```python
from build123d import *

# Parameters (mm, degrees)
BRACKET_PLATE_PROFILE_R    = 9
BRACKET_PLATE_PROFILE_R_2  = 4
BRACKET_PLATE_PROFILE_R_3  = 6
BRACKET_PLATE_8MM_DEPTH    = 8
ARMS_70MM_DEPTH            = 70
GUSSET_TAPER_CUT_PROFILE_R = 6
GUSSET_TAPER_CUT_DEPTH     = 50
ARM_TRIM_CUT_PROFILE_R     = 4
ARM_TRIM_CUT_DEPTH         = 50


with BuildPart() as part:
    # Bracket Plate Profile → Bracket Plate 8mm (new body)
    with BuildSketch(Plane.XY):
        with BuildLine():
            Line((-48.472135955, 36.092742474), (-14.562305899, -10.580134541))
            ThreePointArc((-14.562305899, -10.580134541), (-5.562305899, -17.119017293), (5.562305899, -17.119017293))
            Line((5.562305899, -17.119017293), (85.708203932, 8.92196355))
            ThreePointArc((85.708203932, 8.92196355), (93.852260087, 22.211855326), (82, 32.334641746))
            Line((82, 32.334641746), (8.459892396, 32.334641746))
            ThreePointArc((8.459892396, 32.334641746), (0.445914591, 33.106300041), (-7.273584527, 35.392919854))
            Line((-7.273584527, 35.392919854), (-39.003147253, 48.212495329))
            ThreePointArc((-39.003147253, 48.212495329), (-48.304086029, 45.720316295), (-48.472135955, 36.092742474))
        make_face()
        Circle(BRACKET_PLATE_PROFILE_R, mode=Mode.SUBTRACT)
        with Locations((-42, 40.795024493)):
            Circle(BRACKET_PLATE_PROFILE_R_2, mode=Mode.SUBTRACT)
        with Locations((82, 20.334641746)):
            Circle(BRACKET_PLATE_PROFILE_R_3, mode=Mode.SUBTRACT)
    extrude(amount=BRACKET_PLATE_8MM_DEPTH)

    # Arm Sections 34x6 → Arms 70mm (add)
    with BuildSketch(Plane.XY.offset(8)):
        Polygon((37.898227453, -6.612439485), (43.604566551, -4.758337518), (32.307498994, 30.01046132), (26.601159896, 28.156359354), align=None)
        Polygon((-38.07371599, 21.780545234), (-34.547004477, 16.926443267), (-12.049603456, 33.271761878), (-15.57631497, 38.125863845), align=None)
    extrude(amount=ARMS_70MM_DEPTH)

    # Gusset Taper Cut Profile → Gusset Taper Cut (cut)
    with BuildSketch(Plane(origin=(38.042260652, 12.360679775, 0), x_dir=(0, 0, -1), z_dir=(0.9510565162951532, 0.30901699437494873, 0))):
        with BuildLine():
            Line((-50.49494029, 9.525500165), (-8, 18.558078561))
            Line((-8, 18.558078561), (-78, 18.558078561))
            Line((-78, 18.558078561), (-78, -18))
            Line((-78, -18), (-8, -18))
            Line((-8, -18), (-8, -14.212271044))
            Line((-8, -14.212271044), (-48, -14.212271044))
            ThreePointArc((-48, -14.212271044), (-59.934262744, -3.466612603), (-50.49494029, 9.525500165))
        make_face()
        with Locations(Location((-48, -2.212271044, 0), (0, 0, 90))):
            Circle(GUSSET_TAPER_CUT_PROFILE_R)
    extrude(amount=-GUSSET_TAPER_CUT_DEPTH, mode=Mode.SUBTRACT)

    # Arm Trim Cut Profile → Arm Trim Cut (cut)
    with BuildSketch(Plane(origin=(-23.511410092, 32.360679775, 0), x_dir=(0.8090169943749487, 0.5877852522924716, 0), z_dir=(-0.5877852522924715, 0.8090169943749486, 0))):
        with Locations(Location((-10, -46, 0), (0, 0, 180))):
            Circle(ARM_TRIM_CUT_PROFILE_R)
        with BuildLine():
            Line((9.808316978, -8), (9.218720146, -8))
            Line((9.218720146, -8), (-2.309906432, -48.205098847))
            ThreePointArc((-2.309906432, -48.205098847), (-11.113384808, -53.92214455), (-18, -46))
            Line((-18, -46), (-18, -78))
            Line((-18, -78), (9.808316978, -78))
            Line((9.808316978, -78), (9.808316978, -8))
        make_face()
    extrude(amount=-ARM_TRIM_CUT_DEPTH, mode=Mode.SUBTRACT)


solid = part.part
```
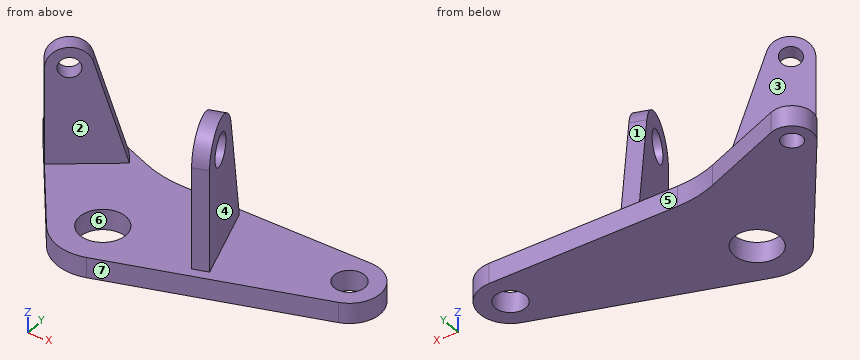
Here's how the part is built. I have some questions about the finished solid (model axes, mm). Face numbers are marked on the shaded views. A direction names the side the tool comes from. Coordinates: 2 decimals unless noted, no trailing zeros. Loops run counter-clockwise (first coordinate to the right, second up) from the corner with the lowest first, then second, coordinate; pieces in that order, holes last. Notation, with made-up numbers: (66, -37.5) - (112, -37.5) arc R20 ccw to (112, -33.5) - close; hole circle Ø4 at (36.25, 22.25). An arc over 180 degrees is marked (long way). Return JSON: item names as keys, results as strings. Group by question number.
Item 1: If we section it at C-C on y = 7.5: State how many separate pieces and enclosed holes the cut face has, and give its area (3 significant figures).
Item 2: I need wall thicknesses on line 1 (Y direction, x = 0, z = 3.5); line 2 (Z direction, x = 2.5, y = -14.5); line 3 (Y direction, x = -42, z = 2.75). Which ranges of each line are inside material? Lowest first, please. Write a range as from..to.
Item 3: If we section it at A-A on z = 35: Write out the boundary of the cut face in (x, y).
Item 4: Will these pins go through, and if not, where does the flat tip stop? P1, Ø1, axis at x = 6.5, y = 1.5, coming from the -Z side; P2, Ø5, axis at y = 13.5, z = 26.5, coming from the -X side; P3, Ø9, axis at x = 45.5, z = 4, coming from the +Y side; P4, Ø5, axis at x = -33, z = 30.5, coming from the +Y side.
Item 5: On a 3-axis mill with a long thin cutter (end or side, diameter ignored), from which of +Z, -Z, +X, -X, +Y, -Y can I reach the whole of each face in a straight line? I mean the marked faces 1, 2, 3 and 4. Say none if no direction works.
Item 6: If we section it at B-B on x = 0: Write out the boundary of the cut face in (y, z), and give its area (3 significant figures).
Item 7: If we section it at D-D on x = 22.5: Write out the boundary of the cut face in (y, z), and give its area (3 significant figures).
Item 8: We'd pull the mould along Y, two halves only. Please class the marked faces 5, 6 and 7: +Y half, -Y half, draft (parallel to the pull), parting line (faces both ways), or undercut.
Calculated:
{
 "1": {"separate pieces": "3", "enclosed holes": "0", "area": "1,050 mm^2"},
 "2": {"line 1": "y = -18..-9, 9..33.2", "line 2": "z = 0..8", "line 3": "y = 27.18..36.8, 44.8..48.8"},
 "3": {"outline": "(-38.07, 21.78) - (-34.55, 16.93) - (-18.79, 28.37) - (-22.32, 33.23) - close; (28.37, 22.7) - (36.73, -3.01) - (42.43, -1.16) - (34.08, 24.55) - close"},
 "4": {"P1": "passes through", "P2": "stops at x = 30.55", "P3": "stops at y = 32.33", "P4": "stops at y = 27.28"},
 "5": {"face 1": "+Z, +Y", "face 2": "+Z, -Y", "face 3": "+Z, -X, +Y", "face 4": "+Z, +X, +Y"},
 "6": {"outline": "(-18, 0) - (-9, 0) - (-9, 8) - (-18, 8) - close; (9, 0) - (33.2, 0) - (33.2, 8) - (9, 8) - close", "area": "266 mm^2"},
 "7": {"outline": "(-11.62, 0) - (32.33, 0) - (32.33, 8) - (-11.62, 8) - close", "area": "352 mm^2"},
 "8": {"face 5": "+Y half", "face 6": "undercut", "face 7": "-Y half"}
}
